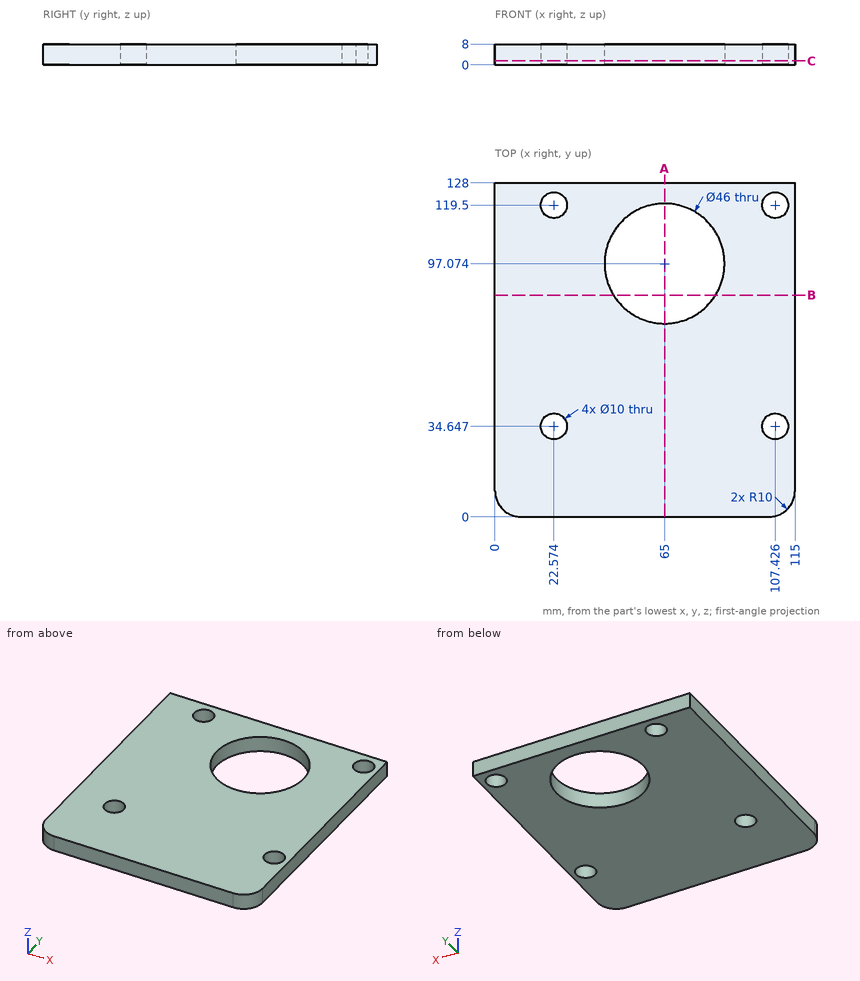
Could you check a few things on this drawing? It's one solid part, dimensions in mm from its lowest x, y, z. Coordinates: 2 decimals unless noted, no trailing zeros. Order: outer loops, then holes, each group sorted by start corner. A loop starts at its lowest first (then second) coordinate and runs counter-clockwise, first axis right, second up. Notation, with made-up numbers: (53, -26.75) - (65, -26.75) arc R17 cw to (65, -7.75) - close; hole circle Ø2 at (-3, 30). An arc over 180 degrees is marked (long way). Answer as a JSON object with one key per item and string values. Group by question number.
Q1. I need wall thicknesses on line 1 (Y direction, x = 24.5, z = 4.75) (1 decimal); line 2 (X direction, y = 108, z = 1.25); line 3 (X direction, y = 113, z = 2.5) (1 decimal). Which ranges of each line are inside material? Lowest first, please. Write a range as from..to.
Q2. Imagine slicing it at C-C (z = 1.5). Please give me the cut outline in (x, y), and give its area (3 significant figures).
Q3. Imagine slicing it at B-B (y = 85). Please give me the cut outline in (x, z), and give its area (3 significant figures).
Q4. Will this pin go through, and if not, where does the flat tip stop? P1, Ø6, axis at x = 22.57, y = 119.5, coming from the -Z side.
Q5. Imagine slicing it at A-A (x = 65). Please give me the cut outline in (y, z).
Determined:
{
 "1": {"line 1": "y = 0..30, 39.3..114.9, 124.1..128", "line 2": "x = 0..44.76, 85.24..115", "line 3": "x = 0..48.4, 81.6..115"},
 "2": {"outline": "(0, 10) arc R10 ccw to (10, 0) - (105, 0) arc R10 ccw to (115, 10) - (115, 128) - (0, 128) - close; hole circle Ø10 at (22.57, 34.65); hole circle Ø10 at (22.57, 119.5); hole circle Ø46 at (65, 97.07); hole circle Ø10 at (107.43, 34.65); hole circle Ø10 at (107.43, 119.5)", "area": "12,700 mm2"},
 "3": {"outline": "(0, 0) - (45.42, 0) - (45.42, 8) - (0, 8) - close; (84.58, 0) - (115, 0) - (115, 8) - (84.58, 8) - close", "area": "607 mm2"},
 "4": {"P1": "passes through"},
 "5": {"outline": "(0, 0) - (74.07, 0) - (74.07, 8) - (0, 8) - close; (120.07, 0) - (128, 0) - (128, 8) - (120.07, 8) - close"}
}
